Verification items for the finished model (mm, model axes). A direction names the side the tool comes from. Give positions to 0.01 mm unless a question says otherwise; leave off trailing zeros. Loops run counter-clockwise (first coordinate to the right, second up) from the corner with the lowest first, then second, coordinate; pieces in that order, holes last. Notation, with made-up numbers: (35, -7) - (44, -7) arc R24 cw to (44, 4) - close; hole circle Ø7 at (29.25, 45.25). An arc over 180 degrees is marked (long way). Answer in a Markdown table with one row per item.
```python
from build123d import *

# Parameters (mm, degrees)
SQUARE_TUBE_30_X_30_X_2_6_15_DEPTH = 600
CUT_EXTRUDE3_DEPTH                 = 113
SKETCH13_R                         = 17.5
CUT_EXTRUDE4_DEPTH                 = 113


with BuildPart() as part:
    # Sketch1 → Square tube 30 X 30 X 2.6(15) (new body)
    with BuildSketch(Plane(origin=(0, 0, 0), x_dir=(0, -1, 0), z_dir=(-1, 0, 0))):
        with BuildLine():
            Line((-21, -15), (21, -15))
            ThreePointArc((21, -15), (23.828427125, -13.828427125), (25, -11))
            Line((25, -11), (25, 11))
            ThreePointArc((25, 11), (23.828427125, 13.828427125), (21, 15))
            Line((21, 15), (-21, 15))
            ThreePointArc((-21, 15), (-23.828427125, 13.828427125), (-25, 11))
            Line((-25, 11), (-25, -11))
            ThreePointArc((-25, -11), (-23.828427125, -13.828427125), (-21, -15))
        make_face()
        with BuildLine():
            Line((-21, -12), (21, -12))
            ThreePointArc((21, -12), (21.707106781, -11.707106781), (22, -11))
            Line((22, -11), (22, 11))
            ThreePointArc((22, 11), (21.707106781, 11.707106781), (21, 12))
            Line((21, 12), (-21, 12))
            ThreePointArc((-21, 12), (-21.707106781, 11.707106781), (-22, 11))
            Line((-22, 11), (-22, -11))
            ThreePointArc((-22, -11), (-21.707106781, -11.707106781), (-21, -12))
        make_face(mode=Mode.SUBTRACT)
    extrude(amount=SQUARE_TUBE_30_X_30_X_2_6_15_DEPTH)

    # Sketch12 → Cut-Extrude3 (cut)
    with BuildSketch(Plane.XZ.offset(25)):
        Polygon((-500, 15), (-494.710190579, -15), (-600, -15), (-600, 15), align=None)
    extrude(amount=-CUT_EXTRUDE3_DEPTH, mode=Mode.SUBTRACT)

    # Sketch13 → Cut-Extrude4 (cut)
    with BuildSketch(Plane.XZ.offset(25)):
        Circle(SKETCH13_R)
    extrude(amount=-CUT_EXTRUDE4_DEPTH, mode=Mode.SUBTRACT)


solid = part.part
```
Q1. Sectioned sample at A-A (y = 12). Record the cut outline in (x, z), and give its area (3 significant figures).
Completed:
| item | result |
|---|---|
| outline | (-500, 15) - (-499.47, 12) - (-12.74, 12) arc R17.5 cw to (-9.01, 15) - close; (-495.24, -12) - (-494.71, -15) - (-9.01, -15) arc R17.5 cw to (-12.74, -12) - close |
| area | 2,920 mm^2 |
Q2. Draft check along Z on faces 3 (the face through (-253, -22, 0)), 4 (the face through (-251, 0, 15)), 5 (the face through (-253, 25, 0)). Enter one of: +Z half, -Z half, draft (parallel to the pull), parting line (faces both ways), or undercut.
Completed:
| item | result |
|---|---|
| face 3 | undercut |
| face 4 | +Z half |
| face 5 | draft |
Q3. Go/stop test with flat-tipped pins: P1, Ø8, axis at y = 15.5, z = 5, coming from the +X side; P2, Ø12, axis at y = 16.5, z = 5, coming from the +X side; P3, Ø12, axis at y = -17, z = 10, coming from the -X side. Record where each tip stops, or that it passes through.
Completed:
| item | result |
|---|---|
| P1 | through |
| P2 | x = -15.86 |
| P3 | x = -500 |
Q4. Tool access check on faces 1 (the face through (-253, 22, 0)), 2 (the face through (-248, 0, -15)). Record the directions out of +Z, -Z, +X, -X, +Y, -Y that give a thin tool (end or side, any length) a straight path to the whole face; none if there is none.
Completed:
| item | result |
|---|---|
| face 1 | +X, -X |
| face 2 | -Z, +X, -X, +Y, -Y |
Q5. Sectioned sample at B-B (x = -271). Record the cut outline in (y, z).
Completed:
| item | result |
|---|---|
| outline | (-25, -11) arc R4 ccw to (-21, -15) - (21, -15) arc R4 ccw to (25, -11) - (25, 11) arc R4 ccw to (21, 15) - (-21, 15) arc R4 ccw to (-25, 11) - close; hole (-22, -11) arc R1 ccw to (-21, -12) - (21, -12) arc R1 ccw to (22, -11) - (22, 11) arc R1 ccw to (21, 12) - (-21, 12) arc R1 ccw to (-22, 11) - close |
Q6. Sectioned sample at C-C (z = -2). Record the cut outline in (x, y).
Completed:
| item | result |
|---|---|
| outline | (-497, -25) - (-17.39, -25) - (-17.39, -22) - (-497, -22) - close; (-497, 22) - (-17.39, 22) - (-17.39, 25) - (-497, 25) - close |
Q7. Thickness scan on line 1 (Y direction, x = -156.5, z = 7.5); line 2 (Z direction, x = -104.5, y = -15.5); line 3 (Y direction, x = -363.5, z = 13). Record the ranges inside material, lowest first.
Completed:
| item | result |
|---|---|
| line 1 | -25 to -22, 22 to 25 |
| line 2 | -15 to -12, 12 to 15 |
| line 3 | -24.46 to 24.46 |
